Input: part model. Units: mm. Frame: model coordinates. A direction names the side the tool comes from. Coordinates: 2 decimals unless noted, no trailing zeros. Order: outer loops, then holes, each group sorted by start corner. A loop starts at its lowest first (then second) coordinate and runs counter-clockwise, first axis right, second up. Notation, with made-up numbers: (-10, 52) -> (3, 52) arc R23 cw to (3, 84) -> close; hole circle Ø9 at (37.25, 43). An arc over 180 degrees is marked (long way). Use one line per item in the form item = value. Start each with the question number.
1) Ray query, line 1 along Y through (x, z) = (1.25, 0); line 2 along X through (y, z) = (76.5, 0); line 3 along Y through (x, z) = (-4.5, -0.5). Return the intervals inside material, ascending.
2) Section query B-B on x = 0. Output: boundary loops of the cut face in (y, z).
3) Draft query along Z for faces 1 (the cylindrical face through (0.07, 37.435, 0.238)), 2 (the cylindrical face through (4.88, 52.7, 1.08)), 3 (the flat face through (0, 125.009, 0)). Return one class per face: pulls with the +Z half, pulls with the -Z half, needs draft (parallel to the pull), parting line crosses it, or undercut.
4) Section query C-C on y = -1. Output: boundary loops of the cut face in (x, z), then the cut area to 3 significant figures.
5) Pin query (flat end, axial travel): pin 1 (4 mm diameter, centred on x = -2, y = 2.5, fed in from +Z); pin 2 (3 mm diameter, centred on x = 4, y = 99.5, fed in from +Z); pin 3 (1 mm diameter, centred on x = -3.5, y = 82, fed in from -Z). Return the tip coordinate at first contact, or that it passes through.
6) Access query for faces 4 (the cylindrical face through (3.905, 7.687, 0.867)), 5 (the cylindrical face through (3.905, 99.659, 0.867)), 6 (the flat face through (0, -14.991, 0)). Directions: +Z, -Z, +X, -X, +Y, -Y. A direction counts if a zero-diameter tool reaches every point of the face in a straight line with its end or side. Return the directions, or none.
7) Section query A-A on y = 55.5. Output: boundary loops of the cut face in (x, z), then the cut area to 3 significant figures.
from build123d import *

# Parameters (mm, degrees)
SKETCH_5_R          = 1.1
CUT_EXTRUDE_1_DEPTH = 10


with BuildPart() as part:
    # 草图4 → 旋转1 (revolve)
    with BuildSketch(Plane.XY, mode=Mode.PRIVATE) as revolve_1_sk:
        Polygon((0, 125.008891803), (4, 125.008891803), (4, 75.008891803), (5, 75.008891803), (5, 31.008891803), (4, 31.008891803), (4, -14.991108197), (0, -14.991108197), align=None)
    revolve(revolve_1_sk.sketch.rotate(Axis((0, 0, 0), (0, 1, 0)), 90), axis=Axis((0, 0, 0), (0, 1, 0)))

    # 草图5 → 切除-拉伸1 (cut, symmetric)
    with BuildSketch(Plane(origin=(0, 0, 0), x_dir=(0, 0, -1), z_dir=(1, 0, 0))):
        with Locations((0, 38.508891803)):
            Circle(SKETCH_5_R)
    extrude(amount=CUT_EXTRUDE_1_DEPTH, both=True, mode=Mode.SUBTRACT)


solid = part.part
Answers below:
q1.line_1 = -14.99 to 37.41, 39.61 to 125.01
q1.line_2 = -4 to 4
q1.line_3 = 31.01 to 37.53, 39.49 to 75.01
q2.outline = (-14.99, -4) -> (31.01, -4) -> (31.01, -5) -> (75.01, -5) -> (75.01, -4) -> (125.01, -4) -> (125.01, 4) -> (75.01, 4) -> (75.01, 5) -> (31.01, 5) -> (31.01, 4) -> (-14.99, 4) -> close; hole circle Ø2.2 at (38.51, 0)
q3.face_1 = undercut
q3.face_2 = parting line crosses it
q3.face_3 = needs draft
q4.outline = circle Ø8 at (0, 0)
q4.area = 50.3 mm^2
q5.pin_1 = 4
q5.pin_2 = 3.12
q5.pin_3 = -2.65
q6.face_4 = -Y
q6.face_5 = +Y
q6.face_6 = +Z, -Z, +X, -X, -Y
q7.outline = circle Ø10 at (0, 0)
q7.area = 78.5 mm^2
